from build123d import *

# Parameters (mm, degrees)
SKETCH_1_R      = 2.5
EXTRUDE_1_DEPTH = 20
SKETCH_2_R      = 5
EXTRUDE_2_DEPTH = 25
SKETCH_3_R      = 7.5
EXTRUDE_3_DEPTH = 2
SKETCH_4_R      = 5
EXTRUDE_4_DEPTH = 15


with BuildPart() as part:
    # 草图1 → 凸台-拉伸1 (new body)
    with BuildSketch(Plane(origin=(0, 0, 0), x_dir=(0, 0, -1), z_dir=(1, 0, 0))):
        Circle(SKETCH_1_R)
    extrude(amount=EXTRUDE_1_DEPTH)

    # 草图2 → 凸台-拉伸2 (add)
    with BuildSketch(Plane.ZY):
        Circle(SKETCH_2_R)
    extrude(amount=EXTRUDE_2_DEPTH)

    # 草图3 → 凸台-拉伸3 (add)
    with BuildSketch(Plane.ZY.offset(25)):
        Circle(SKETCH_3_R)
    extrude(amount=EXTRUDE_3_DEPTH)

    # 草图4 → 凸台-拉伸4 (add)
    with BuildSketch(Plane.ZY.offset(27)):
        Circle(SKETCH_4_R)
    extrude(amount=EXTRUDE_4_DEPTH)


solid = part.part
Source: CAD feature listing. Evaluate the final solid. Frame: model axes, mm. A direction names the side the tool comes from. Give positions to 0.01 mm unless a question says otherwise; leave off trailing zeros. Write each loop counter-clockwise with the first axis right and the second up, starting at its lowest first coordinate (ties: lowest second). Pieces come first, ordered by that corner, then holes. Notation, with made-up numbers: (28.5, 5) -> (55.5, 5) arc R23 cw to (55.5, 13) -> close; hole circle Ø11 at (27.5, -31.5). An arc over 180 degrees is marked (long way). Return JSON: item names as keys, results as strings. Group by question number.
1. Access query for faces 1 (the face through (-34.39, -4.88, -1.08)), 2 (the face through (-42, 0, 0)), 3 (the face through (9.86, -2.44, 0.54)). Directions: +Z, -Z, +X, -X, +Y, -Y. A direction counts if a zero-diameter tool reaches every point of the face in a straight line with its end or side. Return the directions, or none.
2. Section D-D, the plane y = -3.75. Output: boundary loops of the cut face in (x, z), then the cut area to 3 significant figures.
3. Section A-A, the plane y = 0. Output: boundary loops of the cut face in (x, z).
4. Material intervals for line 1 (X direction, y = 2, z = 5.75); line 2 (X direction, y = -2, z = -3.5); line 3 (Y direction, x = 15, z = 1.5), sorted ascending. Write a range as from..to.
5. Section C-C, the plane x = 2.5. Output: boundary loops of the cut face in (y, z), then the cut area to 3 significant figures.
6. Pin query (flat end, axial travel): pin 1 Ø1 at (x, y) = (6.5, -4.5) entering from +Z; pin 2 Ø5 at (x, y) = (13.5, 2) entering from +Z; pin 3 Ø5 at (x, y) = (-3.5, 0.5) entering from +Z; pin 4 Ø2 at (x, z) = (6, 0.5) entering from -Y. Return the tip coordinate at first contact, or that it passes through.
Determined:
{
 "1": {"face 1": "-X", "face 2": "+Z, -Z, -X, +Y, -Y", "face 3": "+X"},
 "2": {"outline": "(-42, -3.31) -> (-27, -3.31) -> (-27, -6.5) -> (-25, -6.5) -> (-25, -3.31) -> (0, -3.31) -> (0, 3.31) -> (-25, 3.31) -> (-25, 6.5) -> (-27, 6.5) -> (-27, 3.31) -> (-42, 3.31) -> close", "area": "291 mm2"},
 "3": {"outline": "(-42, -5) -> (-27, -5) -> (-27, -7.5) -> (-25, -7.5) -> (-25, -5) -> (0, -5) -> (0, -2.5) -> (20, -2.5) -> (20, 2.5) -> (0, 2.5) -> (0, 5) -> (-25, 5) -> (-25, 7.5) -> (-27, 7.5) -> (-27, 5) -> (-42, 5) -> close"},
 "4": {"line 1": "x = -27..-25", "line 2": "x = -42..0", "line 3": "y = -2..2"},
 "5": {"outline": "circle Ø5 at (0, 0)", "area": "19.6 mm2"},
 "6": {"pin 1": "passes through", "pin 2": "stops at z = 2.5", "pin 3": "stops at z = 5", "pin 4": "stops at y = -2.5"}
}
